Part print with two shaded views. Sizes in mm from the minimum x, y, z corner. A direction names the side the tool comes from. Round coordinates to 2 decimals unless told otherwise and drop trailing zeros. Loops run counter-clockwise (first coordinate to the right, second up) from the corner with the lowest first, then second, coordinate; pieces in that order, holes last. Notation, with made-up numbers: (-10, -9.75) - (14, -9.75) arc R17 cw to (14, 22.25) - close; hole circle Ø2 at (67, 34). An arc over 180 degrees is marked (long way). Use a Markdown table: item, result.
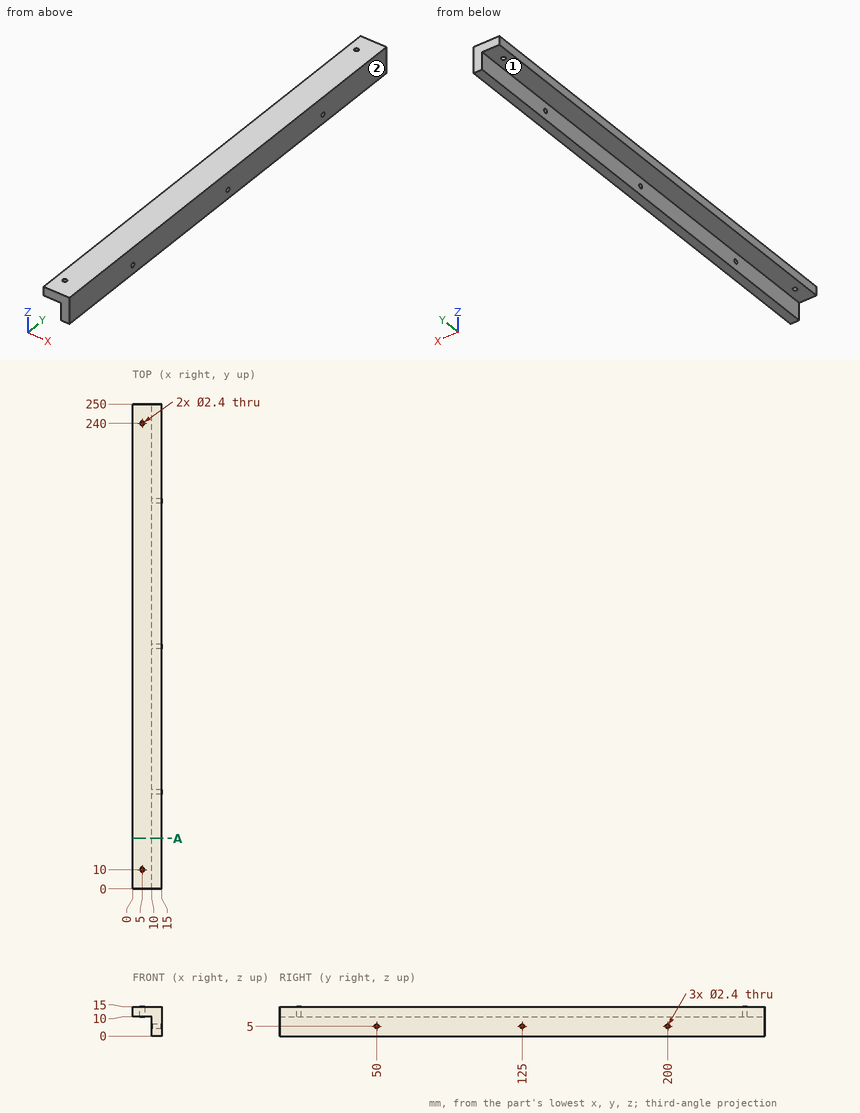
Q1. Cut at A-A, the plane y = 26. List the corners of the cut face in (x, z).
Results found:
| item | result |
|---|---|
| outline | (0, 10) - (10, 10) - (10, 0) - (15, 0) - (15, 15) - (0, 15) - close |
Q2. Which spindle directions (+Z, -Z, +X, -X, +Y, -Y) get a long thin tool onto all of the face, cutting with end or side? Do the marked faces 1 and 2. Say none if no direction does.
Results found:
| item | result |
|---|---|
| face 1 | -Z, -X, +Y, -Y |
| face 2 | +Z, -Z, +X, +Y, -Y |
Q3. Drop flat-ended pins along their axis: pin 1 (1.9 mm diameter, centred on y = 125, z = 5, fed in from -X); pin 2 (8 mm diameter, centred on x = 3.5, y = 138.5, fed in from -Z); pin 3 (4 mm diameter, centred on y = 71.5, z = 2.5, fed in from -X). Give the stop position or say it passes through.
Results found:
| item | result |
|---|---|
| pin 1 | passes through |
| pin 2 | stops at z = 10 |
| pin 3 | stops at x = 10 |
Q4. Probe line 1 (Y direction, x = 4.75, z = 14.25); line 2 (Z direction, x = 11.25, y = 200); line 3 (Y direction, x = 12.75, z = 4). List the from-to ranges inside material, lowest first.
Results found:
| item | result |
|---|---|
| line 1 | y = 0 to 8.83, 11.17 to 238.83, 241.17 to 250 |
| line 2 | z = 0 to 3.8, 6.2 to 15 |
| line 3 | y = 0 to 49.34, 50.66 to 124.34, 125.66 to 199.34, 200.66 to 250 |
